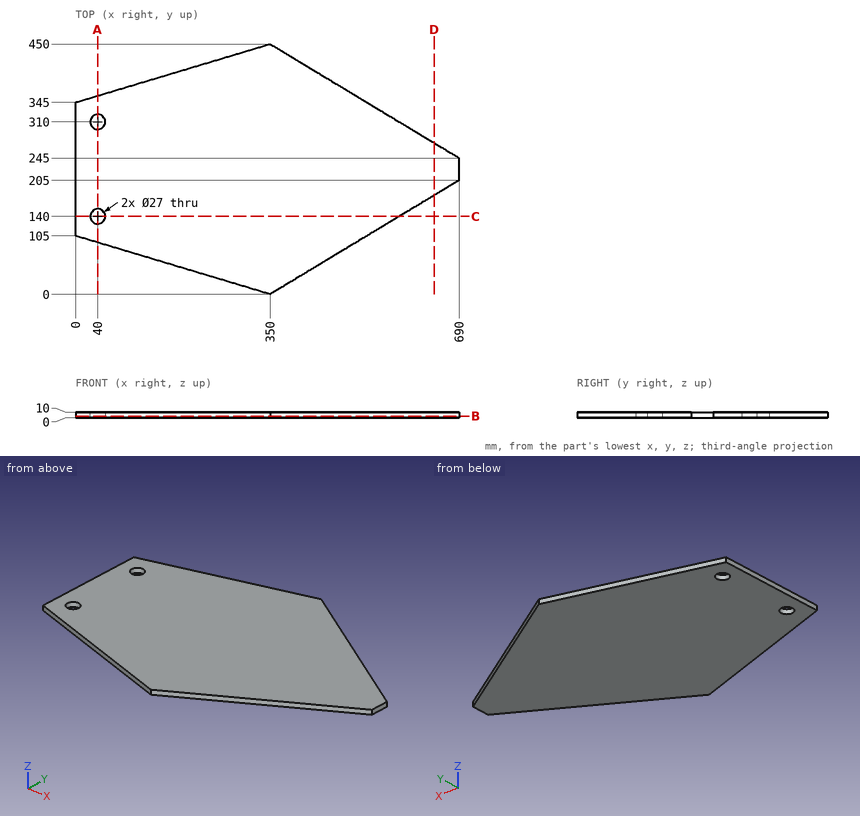
Can you work these out from the drawing? Everything is in mm from the part's minimum corner. Coordinates: 2 decimals unless noted, no trailing zeros. Order: outer loops, then holes, each group sorted by start corner. A loop starts at its lowest first (then second) coordinate and runs counter-clockwise, first axis right, second up. Notation, with made-up numbers: (-15.5, 86) -> (-5.5, 86) arc R6 ccw to (-5.5, 96) -> close; hole circle Ø2 at (84.25, -22). An arc over 180 degrees is marked (long way). Return JSON: item names as keys, results as strings.
1) If we section it at D-D on x = 645: List the corners of the cut face in (y, z) for me.
Conclusion:
{"outline": "(177.87, 0) -> (272.13, 0) -> (272.13, 10) -> (177.87, 10) -> close"}
2) I'm going to push flat-ended pins straight in: P1, Ø1.5, axis at x = 484.5, z = 8.5, coming from the +Y side; P2, Ø16, axis at x = 40, y = 310, coming from the -Z side; P3, Ø5, axis at x = 549, z = 2, coming from the +Y side. Where does each tip first touch, or does it pass through?
Conclusion:
{"P1": "stops at y = 369.36", "P2": "passes through", "P3": "stops at y = 331.52"}
3) If we section it at B-B on z = 3: List the corners of the cut face in (x, y) for me, plus the area to 3 significant figures.
Conclusion:
{"outline": "(0, 105) -> (350, 0) -> (690, 205) -> (690, 245) -> (350, 450) -> (0, 345) -> close; hole circle Ø27 at (40, 140); hole circle Ø27 at (40, 310)", "area": "203,000 mm²"}
4) If I drill on probe 1 along Y at (x, z) = (40, 6.5); probe 2 along X at (y, z) = (176.5, 7.25); probe 3 along Y at (x, z) = (178, 2.75), over which ranges is the centre line in solid material (lowest first)?
Conclusion:
{"probe 1": "y = 93 to 126.5, 153.5 to 296.5, 323.5 to 357", "probe 2": "x = 0 to 642.73", "probe 3": "y = 51.6 to 398.4"}
5) If we section it at A-A on x = 40: List the corners of the cut face in (y, z) for me, plus the area to 3 significant figures.
Conclusion:
{"outline": "(93, 0) -> (126.5, 0) -> (126.5, 10) -> (93, 10) -> close; (153.5, 0) -> (296.5, 0) -> (296.5, 10) -> (153.5, 10) -> close; (323.5, 0) -> (357, 0) -> (357, 10) -> (323.5, 10) -> close", "area": "2,100 mm²"}
6) If we section it at C-C on y = 140: List the corners of the cut face in (x, z) for me, plus the area to 3 significant figures.
Conclusion:
{"outline": "(0, 0) -> (26.5, 0) -> (26.5, 10) -> (0, 10) -> close; (53.5, 0) -> (582.2, 0) -> (582.2, 10) -> (53.5, 10) -> close", "area": "5,550 mm²"}
